```python
from build123d import *

# Parameters (mm, degrees)
SKETCH1_R           = 37.5
SKETCH1_R_2         = 25
SKETCH1_R_3         = 3.5
BOSS_EXTRUDE1_DEPTH = 1


with BuildPart() as part:
    # Sketch1 → Boss-Extrude1 (new body)
    with BuildSketch(Plane.XY):
        Circle(SKETCH1_R)
        Circle(SKETCH1_R_2, mode=Mode.SUBTRACT)
        with Locations((0, 30.5)):
            Circle(SKETCH1_R_3, mode=Mode.SUBTRACT)
        with Locations((30.5, 0)):
            Circle(SKETCH1_R_3, mode=Mode.SUBTRACT)
        with Locations((0, -30.5)):
            Circle(SKETCH1_R_3, mode=Mode.SUBTRACT)
        with Locations((-30.5, 0)):
            Circle(SKETCH1_R_3, mode=Mode.SUBTRACT)
    extrude(amount=BOSS_EXTRUDE1_DEPTH)


solid = part.part
```
For this review, take the finished solid that the model builds, in its own axes (mm). Coordinates: 2 decimals unless noted, no trailing zeros. Write each loop counter-clockwise with the first axis right and the second up, starting at its lowest first coordinate (ties: lowest second). Pieces come first, ordered by that corner, then holes. Notation, with made-up numbers: (60, 10) -> (82, 10) arc R25 cw to (82, 35) -> close; hole circle Ø2 at (-8, 2). An arc over 180 degrees is marked (long way). Put each result on its own line as item: value.
Q1. The part is to be moulded in two halves that separate along Y. For faces 1 (the cylindrical face through (-4.88, 37.18, 0.49)), 2 (the cylindrical face through (33.84, 1.05, 0.49)), 3 (the flat face through (8, -24, 1)), say which applies: +Y half, -Y half, draft (parallel to the pull), parting line (faces both ways), or undercut.
From the geometry:
face 1: parting line
face 2: undercut
face 3: draft
Q2. Take a section at C-C, the plane x = 8.5. State the section outline as (y, z) points.
From the geometry:
outline: (-36.52, 0) -> (-23.51, 0) -> (-23.51, 1) -> (-36.52, 1) -> close; (23.51, 0) -> (36.52, 0) -> (36.52, 1) -> (23.51, 1) -> close
Q3. Take a section at D-D, the plane y = -23.5. State the section outline as (x, z) points, then the cut area to 3 significant figures.
From the geometry:
outline: (-29.22, 0) -> (-8.53, 0) -> (-8.53, 1) -> (-29.22, 1) -> close; (8.53, 0) -> (29.22, 0) -> (29.22, 1) -> (8.53, 1) -> close
area: 41.4 mm2
Q4. Take a section at A-A, the plane x = 0. State the section outline as (y, z) points, then the cut area to 3 significant figures.
From the geometry:
outline: (-37.5, 0) -> (-34, 0) -> (-34, 1) -> (-37.5, 1) -> close; (-27, 0) -> (-25, 0) -> (-25, 1) -> (-27, 1) -> close; (25, 0) -> (27, 0) -> (27, 1) -> (25, 1) -> close; (34, 0) -> (37.5, 0) -> (37.5, 1) -> (34, 1) -> close
area: 11.0 mm2
Q5. Wall thickness on L1, parallel to Y at x = 0, z = 0.5; L2, parallel to X at y = -2.5, z = 0.65; L3, parallel to X at y = -2, z = 0.3: over which ranges is each line inside the solid? List them lowest first.
From the geometry:
L1: y = -37.5 to -34, -27 to -25, 25 to 27, 34 to 37.5
L2: x = -37.42 to -32.95, -28.05 to -24.87, 24.87 to 28.05, 32.95 to 37.42
L3: x = -37.45 to -33.37, -27.63 to -24.92, 24.92 to 27.63, 33.37 to 37.45
